```python
from build123d import *
from OCP.BRepFilletAPI import BRepFilletAPI_MakeChamfer

# Parameters (mm, degrees)
SKETCH_1_R          = 19
EXTRUDE_1_DEPTH     = 16
SKETCH_3_R          = 14
EXTRUDE_2_DEPTH     = 16
SKETCH_4_R          = 19
EXTRUDE_3_DEPTH     = 2.5
SKETCH_5_R          = 11
EXTRUDE_4_DEPTH     = 17
HOLE_WIZARD_1_D     = 9
HOLE_WIZARD_1_DEPTH = 5
SKETCH_7_R          = 4
EXTRUDE_5_DEPTH     = 4
EXTRUDE_6_DEPTH     = 4.3
CUT_EXTRUDE_START   = -2
CUT_EXTRUDE_1_DEPTH = 2
SKETCH_11_W         = 1.8
SKETCH_11_H         = 18.3
EXTRUDE_7_DEPTH     = 13.02
CHAMFER_1_SIZE      = 3
CHAMFER_1_SIZE2     = 5
CHAMFER_2_SIZE      = 5


with BuildPart() as part:
    # 草图1 → 拉伸1 (new body)
    with BuildSketch(Plane.XY):
        Circle(SKETCH_1_R)
    extrude(amount=EXTRUDE_1_DEPTH)

    # 草图3 → 拉伸2 (add)
    with BuildSketch(Plane.XY.offset(16)):
        Circle(SKETCH_3_R)
    extrude(amount=EXTRUDE_2_DEPTH)

    # 草图4 → 拉伸3 (add)
    with BuildSketch(Plane.XY.offset(32)):
        Circle(SKETCH_4_R)
    extrude(amount=EXTRUDE_3_DEPTH)

    # 草图5 → 拉伸4 (add)
    with BuildSketch(Plane.XY.offset(34.5)):
        Circle(SKETCH_5_R)
    extrude(amount=EXTRUDE_4_DEPTH)

    # 孔1
    with Locations(Plane.XY.offset(51.5)):
        with Locations((0, 0)):
            Hole(HOLE_WIZARD_1_D / 2, depth=HOLE_WIZARD_1_DEPTH)

    # 草图7 → 拉伸5 (add)
    with BuildSketch(Plane.XY.offset(46.5)):
        with Locations(Location((0, 0, 0), (0, 0, 180))):
            Circle(SKETCH_7_R)
    extrude(amount=EXTRUDE_5_DEPTH)

    # 草图9 → 拉伸6 (add)
    with BuildSketch(Plane.XY.offset(50.5)):
        with BuildLine():
            Line((-2, 3.464101615), (-2, -3.464101615))
            ThreePointArc((-2, -3.464101615), (0, -4), (2, -3.464101615))
            Line((2, -3.464101615), (2, 3.464101615))
            ThreePointArc((2, 3.464101615), (0, 4), (-2, 3.464101615))
        make_face()
    extrude(amount=EXTRUDE_6_DEPTH)

    # 草图10 → 切除-拉伸1 (cut)
    with BuildSketch(Plane.XY.offset(54.8).offset(CUT_EXTRUDE_START)):
        with BuildLine():
            Line((-0.9, 3.897435054), (-0.9, -3.897435054))
            ThreePointArc((-0.9, -3.897435054), (0, -4), (0.9, -3.897435054))
            Line((0.9, -3.897435054), (0.9, 3.897435054))
            ThreePointArc((0.9, 3.897435054), (0, 4), (-0.9, 3.897435054))
        make_face()
    extrude(amount=CUT_EXTRUDE_1_DEPTH, mode=Mode.SUBTRACT)

    # 草图11 → 拉伸7 (add)
    with BuildSketch(Plane.XY.offset(52.8)):
        Rectangle(SKETCH_11_W, SKETCH_11_H)
    extrude(amount=EXTRUDE_7_DEPTH)

    # 倒角1: one chamfer whose edges measure the first distance from different faces: ONE call of the kernel's chamfer builder (chamfer() names one face for all edges)
    chamfer_1_edges_1 = [part.edges().sort_by_distance(p)[0] for p in [
        (0, 9.15, 65.82),
    ]]
    chamfer_1_side_1 = [part.faces().sort_by_distance(p)[0] for p in [
        (0, 9.15, 59.31),
    ]]
    chamfer_1_edges_2 = [part.edges().sort_by_distance(p)[0] for p in [
        (0, -9.15, 65.82),
    ]]
    chamfer_1_side_2 = [part.faces().sort_by_distance(p)[0] for p in [
        (0, -9.15, 59.31),
    ]]
    chamfer_1 = BRepFilletAPI_MakeChamfer(part.part.solid().wrapped)
    for e in chamfer_1_edges_1:
        chamfer_1.Add(CHAMFER_1_SIZE, CHAMFER_1_SIZE2, e.wrapped, chamfer_1_side_1[0].wrapped)  # the first distance lies on this face
    for e in chamfer_1_edges_2:
        chamfer_1.Add(CHAMFER_1_SIZE, CHAMFER_1_SIZE2, e.wrapped, chamfer_1_side_2[0].wrapped)  # the first distance lies on this face
    add(Compound.cast(chamfer_1.Shape()), mode=Mode.REPLACE)

    # 倒角2
    chamfer_2_edges = [part.edges().sort_by_distance(p)[0] for p in [
        (0, 9.15, 52.8),
        (0, -9.15, 52.8),
    ]]
    chamfer(chamfer_2_edges, length=CHAMFER_2_SIZE)


solid = part.part
```
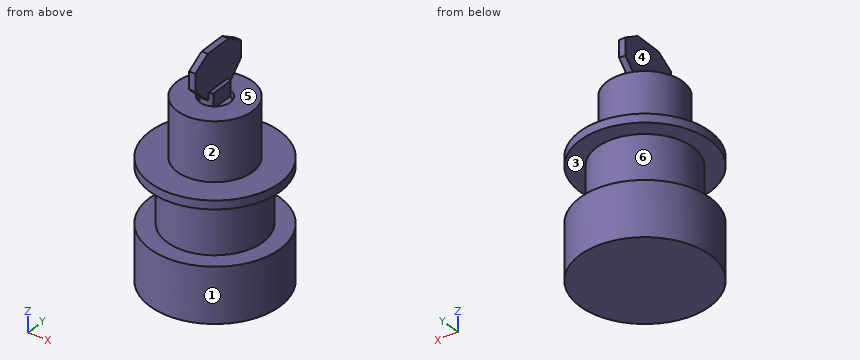
Input: part model. Units: mm. Frame: model coordinates. Face numbers are marked on the shaded views. A direction names the side the tool comes from. Round coordinates to 2 decimals unless told otherwise and drop trailing zeros. Write each loop counter-clockwise with the first axis right and the second up, starting at its lowest first coordinate (ties: lowest second). Pieces come first, ordered by that corner, then holes. Notation, with made-up numbers: (74, 62.5) -> (97, 62.5) arc R23 ccw to (97, 73.5) -> close; hole circle Ø9 at (37, 24.5). An arc over 180 degrees is marked (long way). Answer as CSV lines item,"result".
1. Contact query for flat-ended pins moving along their axis: P1, Ø5, axis at y = -4, z = 22.5, coming from the +X side; P2, Ø1.6, axis at x = -3, y = -1.5, coming from the +Z side; P3, Ø1.5, axis at y = -3, z = 30.5, coming from the -X side; P4, Ø3, axis at x = -2, y = -4, coming from the -Z side. Output: stop coordinate, or through.
Geometry says:
P1,"stops at x = 13.92"
P2,"stops at z = 50.5"
P3,"stops at x = -13.82"
P4,"stops at z = 0"
2. Reachability of the marked faces 1, 2 and 3 from +Z, -Z, +X, -X, +Y, -Y: full face, straight path, thin tool, end or side. Return the list, or none.
Geometry says:
face 1,"+Z, -Z"
face 2,"+Z"
face 3,"none"
3. Section B-B (x = 17). Return the cut outline in (y, z).
Geometry says:
outline,"(-8.49, 0) -> (8.49, 0) -> (8.49, 16) -> (-8.49, 16) -> close; (-8.49, 32) -> (8.49, 32) -> (8.49, 34.5) -> (-8.49, 34.5) -> close"
4. Ray query, L1, parallel to Y at x = 0, z = 49.5; L2, parallel to Z at x = 6, y = 15.5; L3, parallel to Z at x = -3, y = -10. Return the intervals inside material, ascending. Write a range as [from, to].
Geometry says:
L1,"y = [-11, -4.5], [-4, 4], [4.5, 11]"
L2,"z = [0, 16], [32, 34.5]"
L3,"z = [0, 51.5]"
5. Section C-C (y = -15). Return the cut outline in (x, z).
Geometry says:
outline,"(-11.66, 0) -> (11.66, 0) -> (11.66, 16) -> (-11.66, 16) -> close; (-11.66, 32) -> (11.66, 32) -> (11.66, 34.5) -> (-11.66, 34.5) -> close"
6. Mould query, pull axis X, two halves, no side actions, for the marked faces 4, 5 and 6. Classes: +X half, -X half, draft (parallel to the pull), parting line (faces both ways), or undercut.
Geometry says:
face 4,"-X half"
face 5,"draft"
face 6,"parting line"
